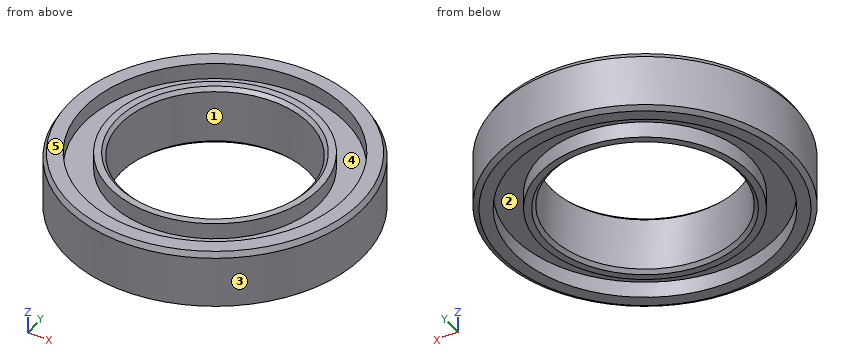
from build123d import *
from OCP.BRepFilletAPI import BRepFilletAPI_MakeChamfer

# Parameters (mm, degrees)
SKETCH1_R           = 42.5
SKETCH1_R_2         = 27
BOSS_EXTRUDE1_DEPTH = 17
SKETCH2_R           = 37.5
SKETCH2_R_2         = 30
CUT_EXTRUDE1_DEPTH  = 4.6
CUT_EXTRUDE2_START  = -4.6
SKETCH3_R           = 37.5
SKETCH3_R_2         = 30
CUT_EXTRUDE2_DEPTH  = 4.6
CHAMFER1_SIZE       = 1.5
CHAMFER1_SIZE2      = 0.866025404
CHAMFER2_SIZE       = 1


with BuildPart() as part:
    # Sketch1 → Boss-Extrude1 (new body)
    with BuildSketch(Plane.XY):
        Circle(SKETCH1_R)
        Circle(SKETCH1_R_2, mode=Mode.SUBTRACT)
    extrude(amount=BOSS_EXTRUDE1_DEPTH)

    # Sketch2 → Cut-Extrude1 (cut)
    with BuildSketch(Plane.XY.offset(17)):
        Circle(SKETCH2_R)
        Circle(SKETCH2_R_2, mode=Mode.SUBTRACT)
    extrude(amount=-CUT_EXTRUDE1_DEPTH, mode=Mode.SUBTRACT)

    # Sketch3 → Cut-Extrude2 (cut)
    with BuildSketch(Plane(origin=(0, 0, 0), x_dir=(-1, 0, 0), z_dir=(0, 0, -1)).offset(CUT_EXTRUDE2_START)):
        with Locations(Location((0, 0, 0), (0, 0, 180))):
            Circle(SKETCH3_R)
        with Locations(Location((0, 0, 0), (0, 0, 180))):
            Circle(SKETCH3_R_2, mode=Mode.SUBTRACT)
    extrude(amount=CUT_EXTRUDE2_DEPTH, mode=Mode.SUBTRACT)

    # Chamfer1: one chamfer whose edges measure the first distance from different faces: ONE call of the kernel's chamfer builder (chamfer() names one face for all edges)
    chamfer1_edges_1 = [part.edges().sort_by_distance(p)[0] for p in [
        (-42.5, 0, 0),
    ]]
    chamfer1_side_1 = [part.faces().sort_by_distance(p)[0] for p in [
        (-41.297918472, 0, 0),
    ]]
    chamfer1_edges_2 = [part.edges().sort_by_distance(p)[0] for p in [
        (-42.5, 0, 17),
    ]]
    chamfer1_side_2 = [part.faces().sort_by_distance(p)[0] for p in [
        (-42.5, 0, 8.5),
    ]]
    chamfer1 = BRepFilletAPI_MakeChamfer(part.part.solid().wrapped)
    for e in chamfer1_edges_1:
        chamfer1.Add(CHAMFER1_SIZE, CHAMFER1_SIZE2, e.wrapped, chamfer1_side_1[0].wrapped)  # the first distance lies on this face
    for e in chamfer1_edges_2:
        chamfer1.Add(CHAMFER1_SIZE, CHAMFER1_SIZE2, e.wrapped, chamfer1_side_2[0].wrapped)  # the first distance lies on this face
    add(Compound.cast(chamfer1.Shape()), mode=Mode.REPLACE)

    # Chamfer2
    chamfer2_edges = [part.edges().sort_by_distance(p)[0] for p in [
        (-27, 0, 0),
        (-27, 0, 17),
    ]]
    chamfer(chamfer2_edges, length=CHAMFER2_SIZE)


solid = part.part
Design review of the part built by this model. Coordinates are the model's own, in mm. Face numbers are marked on the shaded views. A direction names the side the tool comes from. Give positions to 0.01 mm unless a question says otherwise; leave off trailing zeros. Loops run counter-clockwise (first coordinate to the right, second up) from the corner with the lowest first, then second, coordinate; pieces in that order, holes last. Notation, with made-up numbers: M 63,67 L 96,67 A7 cw 96,71 Z; hole C 42.25,-27.75 d8. An arc over 180 degrees is marked long. Answer as a JSON object with one key per item and string values.
Item 1: For P1, Ø4, axis at x = -33.5, z = 14.5, coming from the +Y side; P2, Ø4, axis at y = -9, z = 8, coming from the -X side; P3, Ø8, axis at y = 18, z = 1.5, coming from the -X side, all flat-tipped, find the tip position at first contact; note any pin that passes through.
Output values:
{"P1": "stops at y = 28.53", "P2": "stops at x = -41.92", "P3": "stops at x = -40.13"}
Item 2: Wall thickness on line 1 along Y through (x, z) = (0, 10.75); line 2 along X through (y, z) = (9.5, 1); line 3 along X through (y, z) = (-8.5, 3.75): over which ranges is each line inside the solid? List them lowest first.
Output values:
{"line 1": "y = -42.5 to -27, 27 to 42.5", "line 2": "x = -41.42 to -36.28, -28.46 to -25.27, 25.27 to 28.46, 36.28 to 41.42", "line 3": "x = -41.64 to -36.52, -28.77 to -25.63, 25.63 to 28.77, 36.52 to 41.64"}
Item 3: We need section C-C (z = 2). State the section outline as (x, y) points.
Output values:
{"outline": "C 0,0 d85; C 0,0 d60; hole C 0,0 d75; hole C 0,0 d54"}
Item 4: Machinability: for the marked faces 1 and 2, which of the approach directions +Z, -Z, +X, -X, +Y, -Y give a long, thin tool a straight path to every point of the face, cutting with its end or side? Answer none if there is none.
Output values:
{"face 1": "+Z, -Z", "face 2": "-Z"}
Item 5: Mouldability with a two-part tool opening along X and no side actions: class the marked faces 3, 4 and 5 as pulls with the +X half, pulls with the -X half, needs draft (parallel to the pull), parting line crosses it, or undercut.
Output values:
{"face 3": "parting line crosses it", "face 4": "undercut", "face 5": "needs draft"}
Item 6: We need section D-D (z = 10.25). State the section outline as (x, y) points, and give its area (3 significant figures).
Output values:
{"outline": "C 0,0 d85; hole C 0,0 d54", "area": "3,380 mm2"}
